from build123d import *

# Parameters (mm, degrees)
EXTRUDE_1_DEPTH     = 25
CUT_EXTRUDE_1_DEPTH = 10
CUT_EXTRUDE_2_DEPTH = 10
FILLET_1_R          = 3
FILLET_2_R          = 1
FILLET_3_R          = 3


with BuildPart() as part:
    # 草图9 → 拉伸-薄壁1 (new, symmetric)
    with BuildSketch(Plane.XY):
        Polygon((17, 0), (0, 0), (0, 18), (-2, 18), (-2, -2), (17, -2), align=None)
    extrude(amount=EXTRUDE_1_DEPTH, both=True)

    # 草图10 → 切除-拉伸1 (cut)
    with BuildSketch(Plane(origin=(0, 0, 0), x_dir=(1, 0, 0), z_dir=(0, 1, 0))):
        with BuildLine():
            Line((5.5, 22.15), (12.5, 22.15))
            ThreePointArc((12.5, 22.15), (14.65, 20), (12.5, 17.85))
            Line((12.5, 17.85), (5.5, 17.85))
            ThreePointArc((5.5, 17.85), (3.35, 20), (5.5, 22.15))
        make_face()
        with BuildLine():
            Line((5.5, -22.15), (12.5, -22.15))
            ThreePointArc((12.5, -22.15), (14.65, -20), (12.5, -17.85))
            Line((12.5, -17.85), (5.5, -17.85))
            ThreePointArc((5.5, -17.85), (3.35, -20), (5.5, -22.15))
        make_face()
        with BuildLine():
            Line((5.5, 2.15), (12.5, 2.15))
            ThreePointArc((12.5, 2.15), (14.65, 0), (12.5, -2.15))
            Line((12.5, -2.15), (5.5, -2.15))
            ThreePointArc((5.5, -2.15), (3.35, 0), (5.5, 2.15))
        make_face()
    extrude(amount=-CUT_EXTRUDE_1_DEPTH, mode=Mode.SUBTRACT)

    # 草图11 → 切除-拉伸2 (cut)
    with BuildSketch(Plane(origin=(0, 0, 0), x_dir=(0, 0, -1), z_dir=(1, 0, 0))):
        with BuildLine():
            Line((-10.35, 13), (-10.35, 7))
            ThreePointArc((-10.35, 7), (-12.5, 4.85), (-14.65, 7))
            Line((-14.65, 7), (-14.65, 13))
            ThreePointArc((-14.65, 13), (-12.5, 15.15), (-10.35, 13))
        make_face()
        with BuildLine():
            Line((10.35, 13), (10.35, 7))
            ThreePointArc((10.35, 7), (12.5, 4.85), (14.65, 7))
            Line((14.65, 7), (14.65, 13))
            ThreePointArc((14.65, 13), (12.5, 15.15), (10.35, 13))
        make_face()
    extrude(amount=-CUT_EXTRUDE_2_DEPTH, mode=Mode.SUBTRACT)

    # 圆角1
    fillet_1_edges = [part.edges().sort_by_distance(p)[0] for p in [
        (-1, 18, 25),
        (-1, 18, -25),
        (17, -1, -25),
        (17, -1, 25),
    ]]
    fillet(fillet_1_edges, radius=FILLET_1_R)

    # 圆角2
    fillet_2_edges = [part.edges().sort_by_distance(p)[0] for p in [
        (0, 0, 0),
    ]]
    fillet(fillet_2_edges, radius=FILLET_2_R)

    # 圆角3
    fillet_3_edges = [part.edges().sort_by_distance(p)[0] for p in [
        (-2, -2, 0),
    ]]
    fillet(fillet_3_edges, radius=FILLET_3_R)


solid = part.part
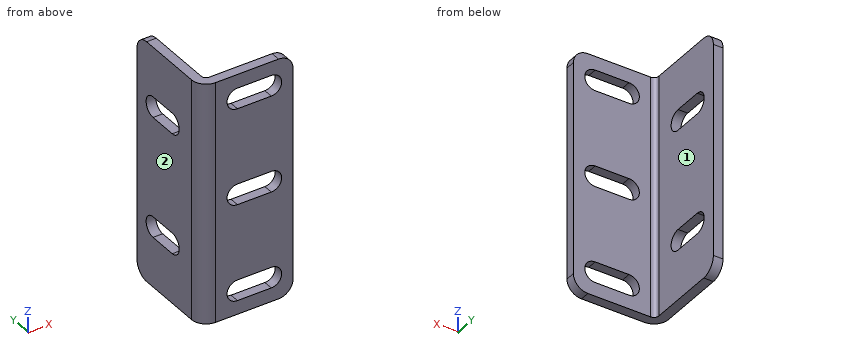
Can you work these out from the model? Positions are in its coordinate system, mm. Face numbers are marked on the shaded views. A direction names the side the tool comes from. Give positions to 0.01 mm unless a question says otherwise; leave off trailing zeros. Write each loop counter-clockwise with the first axis right and the second up, starting at its lowest first coordinate (ties: lowest second). Pieces come first, ordered by that corner, then holes. Notation, with made-up numbers: (27, -6.75) -> (49, -6.75) arc R28 cw to (49, 25.25) -> close; hole circle Ø11 at (30, 54). An arc over 180 degrees is marked (long way). Answer as a JSON object with one key per item and string values. Group by question number.
Item 1: Suppose I cut it at B-B (x = 6.75). Please give me the cut outline in (y, z), plus the area to 3 significant figures.
Item 2: For the marked faces 1 and 2, which set-ups out of +Z, -Z, +X, -X, +Y, -Y let a thin tool reach every point of the face, with its end or its side?
Item 3: Please list where these lines run through material, in increasing order: line 1 (X direction, y = 15.5, z = 1); line 2 (Y direction, x = 0.25, z = 7). Write a range as [from, to].
Item 4: I'm going to push flat-ended pins straight in: P1, Ø8, axis at x = 14.5, z = -12, coming from the +Y side; P2, Ø10, axis at x = 9.5, y = 6.5, coming from the +Z side. Where does each tip first touch, or does it pass through?
Item 5: Suppose I cut it at A-A (z = 12.5). Please give me the cut outline in (x, y).
Item 6: Suppose I cut it at D-D (z = 20). Please give me the cut outline in (x, y).
Item 7: Suppose I cut it at C-C (y = 7.5). Please give me the cut outline in (x, z).
Findings:
{
 "1": {"outline": "(-2, -25) -> (0, -25) -> (0, -22.15) -> (-2, -22.15) -> close; (-2, -17.85) -> (0, -17.85) -> (0, -2.15) -> (-2, -2.15) -> close; (-2, 2.15) -> (0, 2.15) -> (0, 17.85) -> (-2, 17.85) -> close; (-2, 22.15) -> (0, 22.15) -> (0, 25) -> (-2, 25) -> close", "area": "74.2 mm²"},
 "2": {"face 1": "+Z, -Z, +X, +Y", "face 2": "+Z, -Z, -X, +Y, -Y"},
 "3": {"line 1": "x = [-2, 0]", "line 2": "y = [-1.9, 0.34]"},
 "4": {"P1": "stops at y = 0", "P2": "passes through"},
 "5": {"outline": "(-2, 1) arc R3 ccw to (1, -2) -> (17, -2) -> (17, 0) -> (1, 0) arc R1 cw to (0, 1) -> (0, 4.85) -> (-2, 4.85) -> close; (-2, 15.15) -> (0, 15.15) -> (0, 18) -> (-2, 18) -> close"},
 "6": {"outline": "(-2, 1) arc R3 ccw to (1, -2) -> (3.35, -2) -> (3.35, 0) -> (1, 0) arc R1 cw to (0, 1) -> (0, 18) -> (-2, 18) -> close; (14.65, -2) -> (17, -2) -> (17, 0) -> (14.65, 0) -> close"},
 "7": {"outline": "(-2, -25) -> (0, -25) -> (0, -14.65) -> (-2, -14.65) -> close; (-2, -10.35) -> (0, -10.35) -> (0, 10.35) -> (-2, 10.35) -> close; (-2, 14.65) -> (0, 14.65) -> (0, 25) -> (-2, 25) -> close"}
}
